Could you check a few things on this model? Use its own coordinates, in mm. Face numbers are marked on the shaded views. A direction names the side the tool comes from. Coordinates: 2 decimals unless noted, no trailing zeros. Loops run counter-clockwise (first coordinate to the right, second up) from the corner with the lowest first, then second, coordinate; pieces in that order, holes last. Notation, with made-up numbers: (45, 74) - (67, 74) arc R19 cw to (67, 86) - close; hole circle Ø4 at (-13.75, 60.25). An arc over 180 degrees is marked (long way). Use CSV: the item, a comma, the result in double quotes.
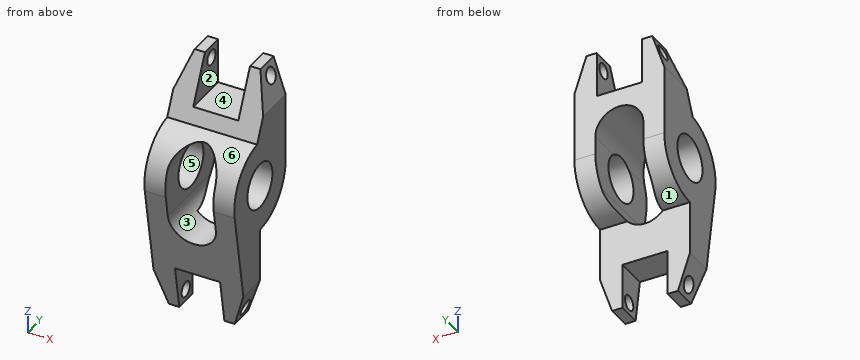
from build123d import *
from OCP.BRepFilletAPI import BRepFilletAPI_MakeChamfer

# Parameters (mm, degrees)
ROCKER_ARM_PROFILE_SKETCH_R  = 4.765
ROCKER_ARM_BODY_DEPTH        = 9.5
END_CHAMFER_2_54X7_62_SIZE   = 2.54
END_CHAMFER_2_54X7_62_SIZE2  = 7.62
END_CHAMFER_7_62X2_54_SIZE   = 7.62
END_CHAMFER_7_62X2_54_SIZE2  = 2.54
HUB_CUT_DEPTH                = 32.656529342
HUB_CUT_DEPTH_BACK           = 32.656529342
FORK_SLOT_CUT_DEPTH          = 32.656529403
FORK_SLOT_CUT_DEPTH_BACK     = 32.656529403
FORK_SLOT_SKETCH_W           = 9.53
FORK_SLOT_SKETCH_H           = 9.53
PIN_HOLES_2X_3_18_DEPTH      = 32.656529403
PIN_HOLES_2X_3_18_DEPTH_BACK = 32.656529403
PIN_HOLES_SKETCH_R           = 1.59


with BuildPart() as part:
    # Rocker Arm Profile Sketch → Rocker Arm Body (new, symmetric)
    with BuildSketch(Plane(origin=(0, 0, 0), x_dir=(0, 0, -1), z_dir=(1, 0, 0))):
        with BuildLine():
            ThreePointArc((9.765, 0), (6.904897718, 6.904897718), (0, 9.765))
            Line((0, 9.765), (-22.23, 9.765))
            Line((-22.23, 9.765), (-22.23, 4.765))
            Line((-22.23, 4.765), (-9.705624325, -1.075212291))
            ThreePointArc((-9.705624325, -1.075212291), (-5.872128035, -7.802136716), (1.653013564, -9.624072483))
            Line((1.653013564, -9.624072483), (28.575, -5))
            Line((28.575, -5), (28.575, 0))
            Line((28.575, 0), (9.765, 0))
        make_face()
        Circle(ROCKER_ARM_PROFILE_SKETCH_R, mode=Mode.SUBTRACT)
    extrude(amount=ROCKER_ARM_BODY_DEPTH, both=True)

    # End Chamfer 2.54x7.62: one chamfer whose edges measure the first distance from different faces: ONE call of the kernel's chamfer builder (chamfer() names one face for all edges)
    end_chamfer_2_54x7_62_edges_1 = [part.edges().sort_by_distance(p)[0] for p in [
        (-9.5, -2.5, -28.575),
    ]]
    end_chamfer_2_54x7_62_side_1 = [part.faces().sort_by_distance(p)[0] for p in [
        (0, -2.5, -28.575),
    ]]
    end_chamfer_2_54x7_62_edges_2 = [part.edges().sort_by_distance(p)[0] for p in [
        (9.5, 7.265, 22.23),
    ]]
    end_chamfer_2_54x7_62_side_2 = [part.faces().sort_by_distance(p)[0] for p in [
        (0, 7.265, 22.23),
    ]]
    end_chamfer_2_54x7_62 = BRepFilletAPI_MakeChamfer(part.part.solid().wrapped)
    for e in end_chamfer_2_54x7_62_edges_1:
        end_chamfer_2_54x7_62.Add(END_CHAMFER_2_54X7_62_SIZE, END_CHAMFER_2_54X7_62_SIZE2, e.wrapped, end_chamfer_2_54x7_62_side_1[0].wrapped)  # the first distance lies on this face
    for e in end_chamfer_2_54x7_62_edges_2:
        end_chamfer_2_54x7_62.Add(END_CHAMFER_2_54X7_62_SIZE, END_CHAMFER_2_54X7_62_SIZE2, e.wrapped, end_chamfer_2_54x7_62_side_2[0].wrapped)  # the first distance lies on this face
    add(Compound.cast(end_chamfer_2_54x7_62.Shape()), mode=Mode.REPLACE)

    # End Chamfer 7.62x2.54: one chamfer whose edges measure the first distance from different faces: ONE call of the kernel's chamfer builder (chamfer() names one face for all edges)
    end_chamfer_7_62x2_54_edges_1 = [part.edges().sort_by_distance(p)[0] for p in [
        (-9.5, 7.265, 22.23),
    ]]
    end_chamfer_7_62x2_54_side_1 = [part.faces().sort_by_distance(p)[0] for p in [
        (-9.5, -0.473958345, -15.36),
    ]]
    end_chamfer_7_62x2_54_edges_2 = [part.edges().sort_by_distance(p)[0] for p in [
        (9.5, -2.5, -28.575),
    ]]
    end_chamfer_7_62x2_54_side_2 = [part.faces().sort_by_distance(p)[0] for p in [
        (9.5, 9.291041655, 7.305),
    ]]
    end_chamfer_7_62x2_54 = BRepFilletAPI_MakeChamfer(part.part.solid().wrapped)
    for e in end_chamfer_7_62x2_54_edges_1:
        end_chamfer_7_62x2_54.Add(END_CHAMFER_7_62X2_54_SIZE, END_CHAMFER_7_62X2_54_SIZE2, e.wrapped, end_chamfer_7_62x2_54_side_1[0].wrapped)  # the first distance lies on this face
    for e in end_chamfer_7_62x2_54_edges_2:
        end_chamfer_7_62x2_54.Add(END_CHAMFER_7_62X2_54_SIZE, END_CHAMFER_7_62X2_54_SIZE2, e.wrapped, end_chamfer_7_62x2_54_side_2[0].wrapped)  # the first distance lies on this face
    add(Compound.cast(end_chamfer_7_62x2_54.Shape()), mode=Mode.REPLACE)

    # Hub Cut Sketch → Hub Cut (cut, two sides: drawn at the far end of the back side and taken through both)
    with BuildSketch(Plane(origin=(0, 0, 0), x_dir=(1, 0, 0), z_dir=(0, 1, 0)).offset(-HUB_CUT_DEPTH_BACK)):
        with BuildLine():
            Line((-5.08, -3.81), (-5.08, 6.35))
            ThreePointArc((-5.08, 6.35), (0, 11.43), (5.08, 6.35))
            Line((5.08, 6.35), (5.08, -3.81))
            ThreePointArc((5.08, -3.81), (0, -8.89), (-5.08, -3.81))
        make_face()
    extrude(amount=HUB_CUT_DEPTH + HUB_CUT_DEPTH_BACK, mode=Mode.SUBTRACT)

    # Fork Slot Sketch → Fork Slot Cut (cut, two sides: drawn at the far end of the back side and taken through both)
    with BuildSketch(Plane(origin=(0, 0, 0), x_dir=(1, 0, 0), z_dir=(0, 1, 0)).offset(-FORK_SLOT_CUT_DEPTH_BACK)):
        with Locations((0, 23.81)):
            Rectangle(FORK_SLOT_SKETCH_W, FORK_SLOT_SKETCH_H)
        with Locations((0, -17.465)):
            Rectangle(FORK_SLOT_SKETCH_W, FORK_SLOT_SKETCH_H)
    extrude(amount=FORK_SLOT_CUT_DEPTH + FORK_SLOT_CUT_DEPTH_BACK, mode=Mode.SUBTRACT)

    # Pin Holes Sketch → Pin Holes 2xØ3.18 (cut, two sides: drawn at the far end of the back side and taken through both)
    with BuildSketch(Plane(origin=(0, 0, 0), x_dir=(0, 0, -1), z_dir=(1, 0, 0)).offset(-PIN_HOLES_2X_3_18_DEPTH_BACK)):
        with Locations(Location((-19.69, 7.225, 0), (0, 0, 180))):
            Circle(PIN_HOLES_SKETCH_R)
        with Locations((26.035, -2.54)):
            Circle(PIN_HOLES_SKETCH_R)
    extrude(amount=PIN_HOLES_2X_3_18_DEPTH + PIN_HOLES_2X_3_18_DEPTH_BACK, mode=Mode.SUBTRACT)


solid = part.part
(1) Please list where these lines run through material, in increasing order: line 1 (X direction, y = -5.5, z = -3); line 2 (Z direction, x = -6.8, y = -2.54) (3 decimals); line 3 (Y direction, x = 6, z = 0) (3 decimals).
Computed:
line 1,"x = -9.5 to -5.08, 5.08 to 9.5"
line 2,"z = -28.575 to -27.625, -24.445 to -4.032, 4.032 to 9.429"
line 3,"y = -9.765 to -4.765, 4.765 to 9.765"
(2) Suppose I cut it at C-C (y = -2). State how many separate pieces and enclosed holes the cut face has, plus the area to 3 significant figures.
Computed:
separate pieces,"4"
enclosed holes,"0"
area,"335 mm²"
(3) Will these pins go through, and if not, where does the flat tip stop? pin 1 (1.9 mm diameter, centred on y = -2.54, z = -26.035, fed in from +X); pin 2 (10 mm diameter, centred on x = -7, y = -4, fed in from +Z); pin 3 (3 mm diameter, centred on y = 4.5, z = 16.5, fed in from -X); pin 4 (5.5 mm diameter, centred on x = -1, y = -3, fed in from -Z) (3 decimals).
Computed:
pin 1,"passes through"
pin 2,"stops at z = 14.16"
pin 3,"stops at x = -9.37"
pin 4,"stops at z = -19.045"
(4) Which directions (+Z, -Z, +X, -X, +Y, -Y) give clear straight access to the entire face, cutting with the end or side of a thin tool? Please do the marked faces 1, 2 and 3.
Computed:
face 1,"-Z, +X, -X, +Y"
face 2,"+Z, +Y, -Y"
face 3,"+Y, -Y"
(5) Thinking about a two-plate mould opening in Y: for the marked faces 4, 5 and 6, which applies, +Y half, -Y half, draft (parallel to the pull), parting line (faces both ways), or undercut?
Computed:
face 4,"draft"
face 5,"undercut"
face 6,"-Y half"
(6) Suppose I cut it at A-A (z = -0.5). Write out the boundary of the cut face in (x, y).
Computed:
outline,"(-9.5, -9.75) - (-5.08, -9.75) - (-5.08, -4.74) - (-9.5, -4.74) - close; (-9.5, 4.74) - (-5.08, 4.74) - (-5.08, 9.75) - (-9.5, 9.75) - close; (5.08, -9.75) - (9.5, -9.75) - (9.5, -4.74) - (5.08, -4.74) - close; (5.08, 4.74) - (9.5, 4.74) - (9.5, 9.75) - (5.08, 9.75) - close"
(7) Suppose I cut it at D-D (z = 7.5). Write out the boundary of the cut face in (x, y) (3 decimals).
Computed:
outline,"(-9.5, -6.253) - (-3.491, -6.253) - (-3.491, 9.765) - (-9.5, 9.765) - close; (3.491, -6.253) - (9.5, -6.253) - (9.5, 9.765) - (3.491, 9.765) - close"
(8) Suppose I cut it at B-B (x = 0). Write out the boundary of the cut face in (y, z) (3 decimals).
Computed:
outline,"(-7.945, -11.43) - (-6.637, -19.045) - (0, -19.045) - (0, -11.43) - close; (-4.04, 8.89) - (9.765, 8.89) - (9.765, 12.7) - (0.321, 12.7) - (-1.075, 9.706) arc R9.765 ccw to start"
